Source: three-view drawing plus pictorial views. Frame: mm from the lowest corner of the part. Give positions to 0.01 mm unless a question says otherwise; leave off trailing zeros. Order: outer loops, then holes, each group sorted by start corner. A loop starts at its lowest first (then second) coordinate and runs counter-clockwise, first axis right, second up. Notation, with made-up numbers: M 47.5,71.25 L 58.5,71.25 A16 cw 58.5,94.25 Z; hole C 85.25,33.25 d5. An arc over 180 degrees is marked long. Use CSV: the item, a comma, the result in double quotes. Start each with the question number.
Item 1: Section query B-B on x = 32.5. Return loops of the section in (y, z).
Item 2: First-contact query: pin 1 (4.5 mm diameter, centred on x = 182.5, z = 82.5, fed in from -Y). Flat tip, straight axial feed; report the tip coordinate or a pass-through.
Item 3: Section query A-A on z = 82.5. Return loops of the section in (x, y), and give its area (3 significant figures).
Item 4: Ray query, probe 1 along Z at (x, y) = (32.5, 12.5); probe 2 along X at (y, z) = (21.75, 82.5). Return the intervals inside material, ascending. Write a range as from..to.
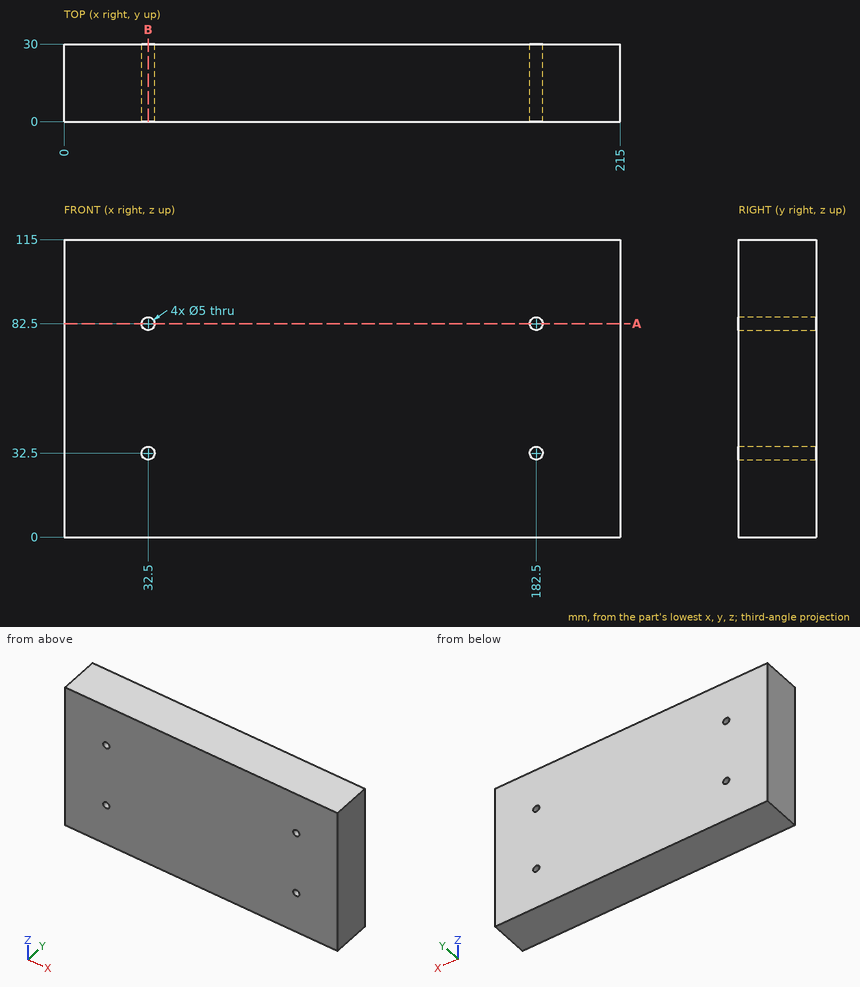
Verdict:
1,outline,"M 0,0 L 30,0 L 30,30 L 0,30 Z; M 0,35 L 30,35 L 30,80 L 0,80 Z; M 0,85 L 30,85 L 30,115 L 0,115 Z"
2,pin 1,"through"
3,outline,"M 0,0 L 30,0 L 30,30 L 0,30 Z; M 35,0 L 180,0 L 180,30 L 35,30 Z; M 185,0 L 215,0 L 215,30 L 185,30 Z"
3,area,"6,150 mm2"
4,probe 1,"0..30, 35..80, 85..115"
4,probe 2,"0..30, 35..180, 185..215"
